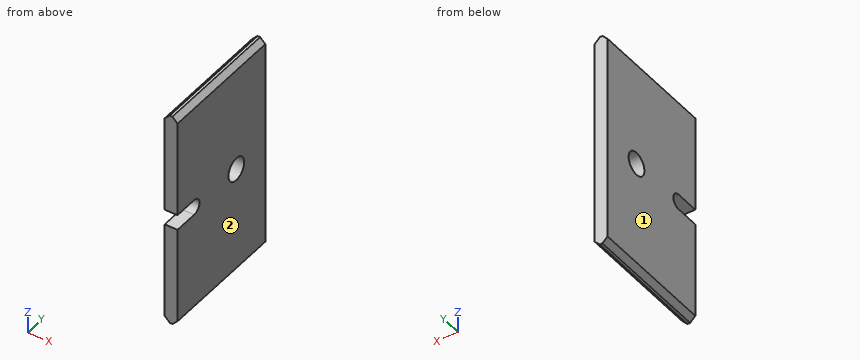
```python
from build123d import *

# Parameters (mm, degrees)
SKETCH1_R           = 45
BOSS_EXTRUDE1_DEPTH = 25
CHAMFER1_SIZE       = 20


with BuildPart() as part:
    # Sketch1 → Boss-Extrude1 (new, symmetric)
    with BuildSketch(Plane(origin=(0, 0, 0), x_dir=(0, 0, -1), z_dir=(1, 0, 0))):
        with BuildLine():
            Line((425, -250), (30, -250))
            Line((30, -250), (30, -155))
            ThreePointArc((30, -155), (0, -125), (-30, -155))
            Line((-30, -155), (-30, -250))
            Line((-30, -250), (-425, -250))
            Line((-425, -250), (-425, 250))
            Line((-425, 250), (425, 250))
            Line((425, 250), (425, -250))
        make_face()
        with Locations((0, 85)):
            Circle(SKETCH1_R, mode=Mode.SUBTRACT)
    extrude(amount=BOSS_EXTRUDE1_DEPTH, both=True)

    # Chamfer1
    chamfer1_edges = [part.edges().sort_by_distance(p)[0] for p in [
        (-25, 0, 425),
        (25, 0, -425),
        (25, 0, 425),
        (-25, 0, -425),
    ]]
    chamfer(chamfer1_edges, length=CHAMFER1_SIZE)


solid = part.part
```
Source: CAD feature listing. Evaluate the final solid. Frame: model axes, mm. Face numbers are marked on the shaded views. Give positions to 0.01 mm unless a question says otherwise; leave off trailing zeros. Loops run counter-clockwise (first coordinate to the right, second up) from the corner with the lowest first, then second, coordinate; pieces in that order, holes last. Notation, with made-up numbers: (86, 73.25) -> (132, 73.25) arc R19 cw to (132, 83.25) -> close; hole circle Ø6 at (6, -38.5). An arc over 180 degrees is marked (long way). Use a Markdown table: item, result. Add a question column.
(1) Ray query, line 1 (Y direction, x = 14, z = 0); line 2 (Z direction, x = -19.5, y = 106.5); line 3 (Y direction, x = 5.5, z = 30.5). Return the intervals inside material, ascending.
(2) First-contact query: pin 1 Ø8 at (x, y) = (14.5, 30.5) entering from -Z; pin 2 Ø10 at (x, y) = (-12, -15) entering from +Z. Flat tips, straight axial feed; report the tip coordinate or a pass-through.
(3) Section query A-A (y = 85). Output: boundary loops of the cut face in (x, z), then the cut area to 3 significant figures.
(4) Section query B-B (z = 0). Output: boundary loops of the cut face in (x, y), then the cut area to 4 significant figures.
(5) Section query C-C (y = -46). Output: boundary loops of the cut face in (x, z).
(6) Pull-direction query (X, two-part tool) for the marked faces 1 and 2; classes: +X half, -X half, draft (parallel to the pull), parting line (faces both ways), or undercut.
Checked values:
| question | item | result |
|---|---|---|
| 1 | line 1 | -125 to 40, 130 to 250 |
| 1 | line 2 | -410.5 to -39.53, 39.53 to 410.5 |
| 1 | line 3 | -250 to 51.91, 118.09 to 250 |
| 2 | pin 1 | z = -419.5 |
| 2 | pin 2 | z = 423 |
| 3 | outline | (-25, -405) -> (-5, -425) -> (5, -425) -> (25, -405) -> (25, -45) -> (-25, -45) -> close; (-25, 45) -> (25, 45) -> (25, 405) -> (5, 425) -> (-5, 425) -> (-25, 405) -> close |
| 3 | area | 37,200 mm^2 |
| 4 | outline | (-25, -125) -> (25, -125) -> (25, 40) -> (-25, 40) -> close; (-25, 130) -> (25, 130) -> (25, 250) -> (-25, 250) -> close |
| 4 | area | 14,250 mm^2 |
| 5 | outline | (-25, -405) -> (-5, -425) -> (5, -425) -> (25, -405) -> (25, 405) -> (5, 425) -> (-5, 425) -> (-25, 405) -> close |
| 6 | face 1 | -X half |
| 6 | face 2 | +X half |
